Model file for the job. Use its own axes, mm. A direction names the side the tool comes from. Give positions to 0.01 mm unless a question says otherwise; leave off trailing zeros. Order: outer loops, then holes, each group sorted by start corner. A loop starts at its lowest first (then second) coordinate and runs counter-clockwise, first axis right, second up. Notation, with made-up numbers: M 0,-33.75 L 7,-33.75 A27 ccw 7,0.25 Z; hole C 41,43.25 d1. An arc over 180 degrees is marked long. Return JSON: item names as keys, results as strings. Group by question number.
1. 3-axis set-ups, long thin cutter, end or side, ignore diameter. For faces 4 (the face through (-48.794, 14.79, 25.379)), 5 (the face through (-69.054, 18.525, -1.277)): which of +Z, -Z, +X, -X, +Y, -Y reach the whole face in a straight line?
2. Slice it at A-A on z = -30.5. List the corners of the cut face in (x, y), then the cut area to 3 significant figures.
3. Wall check: probe 1 along Z at (x, y) = (-7.5, 28.5); probe 2 along X at (y, z) = (16.25, 65); probe 3 along X at (y, z) = (19.25, -42). Give the ranges that are in metal, low to high. Write a range as [from, to].
4. Pin check, flat tips, straight feed: pin 1 (1 mm diameter, centred on y = 20, z = -36, fed in from +X); pin 2 (12 mm diameter, centred on x = 39, y = 24, fed in from -Z); pin 3 (1.5 mm diameter, centred on y = 5.5, z = -31, fed in from -X). Stop position of each tip, or through.
5. Slice it at B-B on x = 15. List the corners of the cut face in (y, z).
6. Two-plate mould, pull along Z, no slides. Class faces 1 (the face through (-52, 30, -19)), 2 (the face through (-78.1, 14.79, -17.34)), 3 (the face through (-1.96, 18.53, 68.77)): released by +Z, released by -Z, zero draft, split by the parting line, or undercut.
from build123d import *

# Parameters (mm, degrees)
SKETCH1_R                    = 80
SKETCH1_R_2                  = 55
BOSS_EXTRUDE1_DEPTH          = 30
M10_TAPPED_HOLE1_D           = 8.5
M10_TAPPED_HOLE1_DEPTH       = 22
M10_TAPPED_HOLE1_CSINK_D     = 10.05
M10_TAPPED_HOLE1_CSINK_ANGLE = 100
M10_TAPPED_HOLE1_TIP         = 2.553657631


with BuildPart() as part:
    # Sketch1 → Boss-Extrude1 (new body)
    with BuildSketch(Plane(origin=(0, 0, 0), x_dir=(1, 0, 0), z_dir=(0, 1, 0))):
        with Locations(Location((0, 0, 0), (0, 0, 270))):
            Circle(SKETCH1_R)
        with Locations(Location((0, 0, 0), (0, 0, 270))):
            Circle(SKETCH1_R_2, mode=Mode.SUBTRACT)
    extrude(amount=BOSS_EXTRUDE1_DEPTH)

    # M10 Tapped Hole1
    with Locations(Plane(origin=(0, 30, 0), x_dir=(1, 0, 0), z_dir=(0, 1, 0))):
        with Locations((0, 65), (65, 0), (0, -65), (-65, 0)):
            CounterSinkHole(M10_TAPPED_HOLE1_D / 2, M10_TAPPED_HOLE1_CSINK_D / 2, depth=M10_TAPPED_HOLE1_DEPTH, counter_sink_angle=M10_TAPPED_HOLE1_CSINK_ANGLE)
            with Locations((0, 0, -(M10_TAPPED_HOLE1_DEPTH + M10_TAPPED_HOLE1_TIP / 2))):  # 118° drill point
                Cone(0, M10_TAPPED_HOLE1_D / 2, M10_TAPPED_HOLE1_TIP, mode=Mode.SUBTRACT)


solid = part.part
Result:
{
 "1": {"face 4": "+Y, -Y", "face 5": "+Y"},
 "2": {"outline": "M -73.96,0 L -45.77,0 L -45.77,30 L -73.96,30 Z; M 45.77,0 L 73.96,0 L 73.96,30 L 45.77,30 Z", "area": "1,690 mm2"},
 "3": {"probe 1": "z = [-79.65, -54.49], [54.49, 79.65]", "probe 2": "x = [-46.64, -4.25], [4.25, 46.64]", "probe 3": "x = [-68.09, -35.51], [35.51, 68.09]"},
 "4": {"pin 1": "stops at x = 71.69", "pin 2": "stops at z = -72.88", "pin 3": "stops at x = -74.06"},
 "5": {"outline": "M 0,-78.58 L 30,-78.58 L 30,-52.92 L 0,-52.92 Z; M 0,52.92 L 30,52.92 L 30,78.58 L 0,78.58 Z"},
 "6": {"face 1": "zero draft", "face 2": "split by the parting line", "face 3": "undercut"}
}
